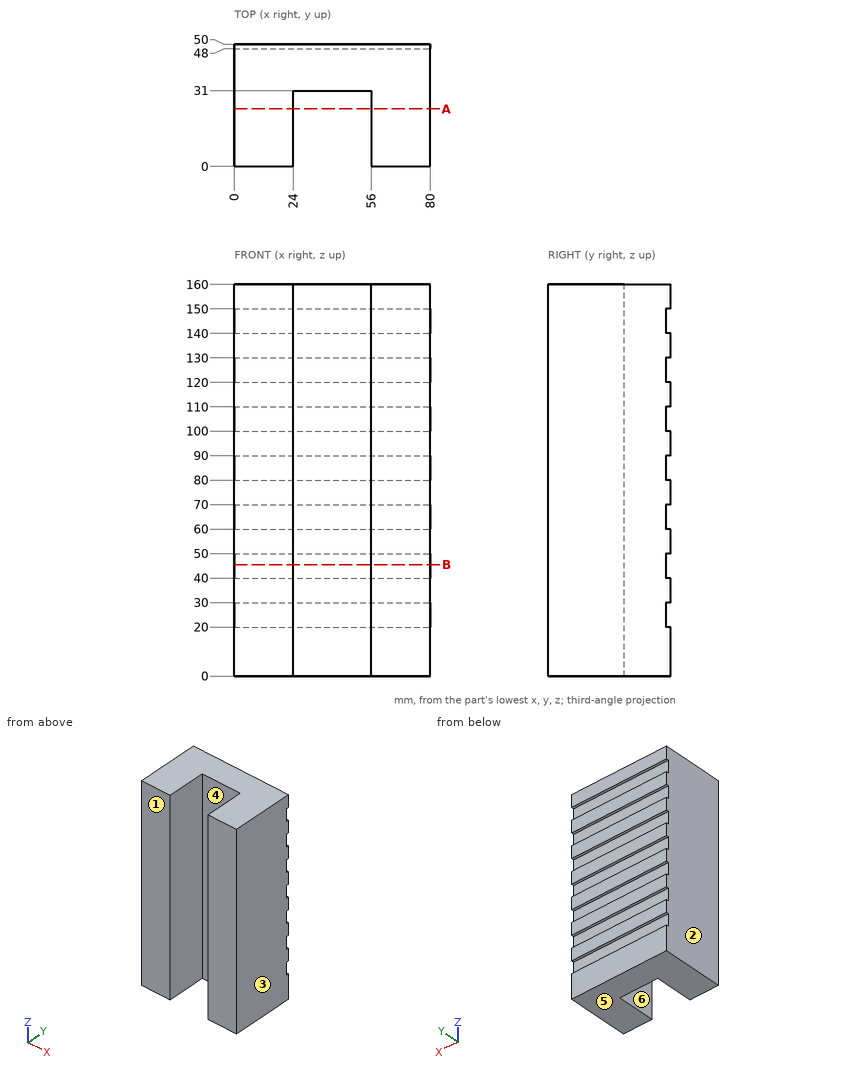
For this review, use the dimensioned drawing (mm, ordinates from the lowest corner) and the shaded views. A direction names the side the tool comes from. Round coordinates to 2 decimals unless told otherwise and drop trailing zeros. Write each loop counter-clockwise with the first axis right and the second up, starting at its lowest first coordinate (ties: lowest second). Pieces come first, ordered by that corner, then holes. Notation, with made-up numbers: (-38.5, -35.5) - (-20.5, -35.5) arc R19 ccw to (-20.5, -21.5) - close; hole circle Ø6 at (-19.5, -2.75). An arc over 180 degrees is marked (long way). One line per item, written item: value. Start each with the question number.
1. The part is to be moulded in two halves that separate along X. For the marked faces 1, 2, 3 and 4, say which applies: released by +X, released by -X, zero draft, split by the parting line, or undercut.
2. Consider section A-A on y = 23.5. Write out the cut boundary in (x, z).
3. Clearance check with flat-ended pins moving along their axes: P1, Ø3, axis at x = 28, z = 25.5, coming from the +Y side; P2, Ø1.5, axis at x = 52.5, z = 142, coming from the -Y side. State where each tip first meets the part, or that it passes through.
4. Machinability: for the marked faces 5 and 6, which of the approach directions +Z, -Z, +X, -X, +Y, -Y give a long, thin tool a straight path to every point of the face, cutting with its end or side? Answer none if there is none.
5. Consider section B-B on z = 45.5. Write out the cut boundary in (x, y).
6. To check wall thickness, follow L1, parallel to X at y = 3, z = 12.5; L2, parallel to Y at x = 61, z = 105.5. State the ranges of each line that lie inside material, in increasing order. Write a range as from..to.
Checks:
1. face 1: zero draft
1. face 2: released by -X
1. face 3: released by +X
1. face 4: undercut
2. outline: (0, 0) - (24, 0) - (24, 160) - (0, 160) - close; (56, 0) - (80, 0) - (80, 160) - (56, 160) - close
3. P1: stops at y = 48
3. P2: stops at y = 31
4. face 5: -Z, +X, -X, +Y, -Y
4. face 6: +Z, -Z, -Y
5. outline: (0, 0) - (24, 0) - (24, 31) - (56, 31) - (56, 0) - (80, 0) - (80, 48) - (0, 48) - close
6. L1: x = 0..24, 56..80
6. L2: y = 0..48
